Input: part model. Units: mm. Frame: model coordinates. Face numbers are marked on the shaded views. A direction names the side the tool comes from. Coordinates: 2 decimals unless noted, no trailing zeros. Write each loop counter-clockwise with the first axis right and the second up, starting at its lowest first coordinate (ties: lowest second). Pieces come first, ordered by that corner, then holes. Notation, with made-up numbers: M 9,-35 L 57,-35 A31 ccw 57,-7 Z; hole C 3,-3 d5. An arc over 180 degrees is marked long. Use one line per item in the form item = value.
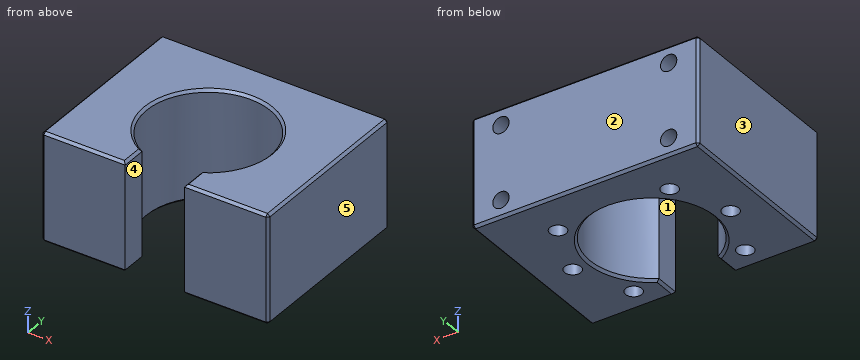
from build123d import *

# Parameters (mm, degrees)
SKETCH_1_W             = 46
SKETCH_1_H             = 36
EXTRUDE_1_DEPTH        = 22
CUT_EXTRUDE_2_DEPTH    = 37.565010598
CHAMFER_1_SIZE         = 0.5
HOLE_WIZARD_M4_1_D     = 3.3
HOLE_WIZARD_M4_1_DEPTH = 12.1
HOLE_WIZARD_M4_1_TIP   = 0.991420021
HOLE_WIZARD_M4_2_D     = 3.3
HOLE_WIZARD_M4_2_DEPTH = 10.1
HOLE_WIZARD_M4_2_TIP   = 0.991420021


with BuildPart() as part:
    # 草图1 → 凸台-拉伸1 (new body)
    with BuildSketch(Plane.XY):
        Rectangle(SKETCH_1_W, SKETCH_1_H)
    extrude(amount=EXTRUDE_1_DEPTH)

    # 草图5 → 切除-拉伸2 (cut, through all)
    with BuildSketch(Plane.XY.offset(22)):
        with BuildLine():
            Line((-6, -12.9658561), (-6, -18))
            Line((-6, -18), (6, -18))
            Line((6, -18), (6, -12.9658561))
            ThreePointArc((6, -12.9658561), (0, 10.5), (-6, -12.9658561))
        make_face()
    extrude(amount=-CUT_EXTRUDE_2_DEPTH, mode=Mode.SUBTRACT)

    # 倒角1
    chamfer_1_edges = [part.edges().sort_by_distance(p)[0] for p in [
        (-23, 0, 22),
        (-14.5, -18, 22),
        (14.5, -18, 0),
        (14.5, -18, 22),
        (0, 10.5, 0),
        (6, -15.48292805, 0),
        (-6, -15.48292805, 0),
        (0, 10.5, 22),
        (-6, -15.48292805, 22),
        (6, -15.48292805, 22),
        (23, 0, 22),
        (-14.5, -18, 0),
        (-23, 0, 0),
        (0, 18, 0),
        (23, 0, 0),
        (0, 18, 22),
        (23, -18, 11),
        (-23, -18, 11),
        (-23, 18, 11),
        (23, 18, 11),
    ]]
    chamfer(chamfer_1_edges, length=CHAMFER_1_SIZE)

    # M4 螺纹孔1
    with Locations(Plane(origin=(0, 18, 0), x_dir=(1, 0, 0), z_dir=(0, 1, 0))):
        with Locations((17, -18.5), (17, -3.5), (-17, -3.5), (-17, -18.5)):
            Hole(HOLE_WIZARD_M4_1_D / 2, depth=HOLE_WIZARD_M4_1_DEPTH)
            with Locations((0, 0, -(HOLE_WIZARD_M4_1_DEPTH + HOLE_WIZARD_M4_1_TIP / 2))):  # 118° drill point
                Cone(0, HOLE_WIZARD_M4_1_D / 2, HOLE_WIZARD_M4_1_TIP, mode=Mode.SUBTRACT)

    # M4 螺纹孔2
    with Locations(Plane(origin=(0, 0, 0), x_dir=(-1, 0, 0), z_dir=(0, 0, -1))):
        with Locations((-16, -2), (-11.313708499, 9.313708499), (11.313708499, 9.313708499), (16, -2), (-11.313708499, -13.313708499), (11.313708499, -13.313708499)):
            Hole(HOLE_WIZARD_M4_2_D / 2, depth=HOLE_WIZARD_M4_2_DEPTH)
            with Locations((0, 0, -(HOLE_WIZARD_M4_2_DEPTH + HOLE_WIZARD_M4_2_TIP / 2))):  # 118° drill point
                Cone(0, HOLE_WIZARD_M4_2_D / 2, HOLE_WIZARD_M4_2_TIP, mode=Mode.SUBTRACT)


solid = part.part
(1) Line query: probe 1 along X at (y, z) = (-2, 5.75); probe 2 along Z at (x, y) = (17, 11.5); probe 3 along X at (y, z) = (-15.5, 11). Output: solid intervals per line, ascending.
Computed:
probe_1 = -23 to -17.65, -14.35 to -12.5, 12.5 to 14.35, 17.65 to 23
probe_2 = 0 to 1.85, 5.15 to 16.85, 20.15 to 22
probe_3 = -23 to -6, 6 to 23
(2) Section query A-A on z = 16. Return the cut outline in (x, y), plus the area to 3 significant figures.
Computed:
outline = M -23,-17.5 L -22.5,-18 L -6,-18 L -6,-12.97 A12.5 cw long 6,-12.97 L 6,-18 L 22.5,-18 L 23,-17.5 L 23,17.5 L 22.5,18 L -22.5,18 L -23,17.5 Z
area = 1,120 mm^2
(3) Set-up query: the marked faces 1 and 2. Return all of +Z, -Z, +X, -X, +Y, -Y with unobstructed straight access to the full face (end or side cutting, diameter ignored); none if empty.
Computed:
face_1 = +Z, -Z, -Y
face_2 = +Z, -Z, +X, -X, +Y
(4) Section query C-C on z = 4.5. State how many separate pieces and enclosed holes the cut face has, plus the area to 3 significant figures.
Computed:
separate_pieces = 1
enclosed_holes = 6
area = 1,000 mm^2
(5) Section query B-B on z = 8.75. Return the cut outline in (x, y), plus the area to 3 significant figures.
Computed:
outline = M -23,-17.5 L -22.5,-18 L -6,-18 L -6,-12.97 A12.5 cw long 6,-12.97 L 6,-18 L 22.5,-18 L 23,-17.5 L 23,17.5 L 22.5,18 L -22.5,18 L -23,17.5 Z; hole C -16,-2 d3.3; hole C -11.31,-13.31 d3.3; hole C -11.31,9.31 d3.3; hole C 11.31,-13.31 d3.3; hole C 11.31,9.31 d3.3; hole C 16,-2 d3.3
area = 1,070 mm^2
(6) First-contact query: pin 1 Ø2 at (x, y) = (8.5, -7) entering from +Z; pin 2 Ø3 at (x, y) = (16, -2) entering from -Z; pin 3 Ø2.5 at (x, z) = (17, 3.5) entering from +Y. Flat tips, straight axial feed; report the tip coordinate or a pass-through.
Computed:
pin_1 = through
pin_2 = 10.19
pin_3 = 5.66
(7) Pull-direction query (X, two-part tool) for the marked faces 3, 4 and 5; classes: pulls with the +X half, pulls with the -X half, needs draft (parallel to the pull), parting line crosses it, or undercut.
Computed:
face_3 = pulls with the -X half
face_4 = undercut
face_5 = pulls with the +X half
